```python
from build123d import *


with BuildPart() as part:
    # Sketch1 → Revolve1 (revolve)
    with BuildSketch(Plane(origin=(0, 0, 0), x_dir=(0, 0, -1), z_dir=(1, 0, 0)), mode=Mode.PRIVATE) as revolve1_sk:
        Polygon((23, 0), (23, 10), (20, 10), (20, 7.5), (10, 7.5), (10, 5), (0, 5), (0, 0), align=None)
    revolve(revolve1_sk.sketch.rotate(Axis((0, 0, 0), (0, 0, -1)), 90), axis=Axis((0, 0, 0), (0, 0, -1)))


solid = part.part
```
For this review, take the finished solid that the model builds, in its own axes (mm). A direction names the side the tool comes from. Round coordinates to 2 decimals unless told otherwise and drop trailing zeros. Write each loop counter-clockwise with the first axis right and the second up, starting at its lowest first coordinate (ties: lowest second). Pieces come first, ordered by that corner, then holes. Notation, with made-up numbers: (35, 40.5) -> (48, 40.5) arc R19 cw to (48, 56.5) -> close; hole circle Ø3 at (44.25, 77). An arc over 180 degrees is marked (long way). One line per question, with ' | ' between items. Start each with the question number.
1) Add section D-D (x = 6.75). Write out the cut boundary in (y, z).
2) Add section A-A (x = 0). Write out the cut boundary in (y, z).
3) Add section C-C (z = -12.25). Write out the cut boundary in (x, y), and give its area (3 significant figures).
4) Machinability: for faces 1 (the cylindrical face through (-10, 0, -21)), 2 (the flat face through (2, 5, -10)), which of the approach directions +Z, -Z, +X, -X, +Y, -Y give a long, thin tool a straight path to every point of the face, cutting with its end or side? Answer none if there is none.
5) Wall thickness on line 1 along Z through (x, y) = (-6.75, 5.25); line 2 along Z through (x, y) = (4, 5); line 3 along X through (y, z) = (1.25, -14.75): over which ranges is each line inside the solid? List them lowest first.
6) For pin 1 Ø6 at (x, y) = (-3, -4.5) entering from +Z; pin 2 Ø1 at (y, z) = (3, -19) entering from +X; pin 3 Ø5 at (x, z) = (-5.5, -14) entering from +Y; pin 4 Ø8 at (x, z) = (-1.5, -14) entering from -Y, all flat-tipped, find the tip position at first contact; note any pin that passes through.
Reported:
1) outline: (-7.38, -23) -> (7.38, -23) -> (7.38, -20) -> (3.27, -20) -> (3.27, -10) -> (-3.27, -10) -> (-3.27, -20) -> (-7.38, -20) -> close
2) outline: (-10, -23) -> (10, -23) -> (10, -20) -> (7.5, -20) -> (7.5, -10) -> (5, -10) -> (5, 0) -> (-5, 0) -> (-5, -10) -> (-7.5, -10) -> (-7.5, -20) -> (-10, -20) -> close
3) outline: circle Ø15 at (0, 0) | area: 177 mm²
4) face 1: +Z, -Z | face 2: +Z
5) line 1: z = -23 to -20 | line 2: z = -23 to -10 | line 3: x = -7.4 to 7.4
6) pin 1: stops at z = 0 | pin 2: stops at x = 7.07 | pin 3: stops at y = 6.87 | pin 4: stops at y = -7.5
